Read the model definition and answer for the solid it produces. Units are mm, in the model's axes. A direction names the side the tool comes from. Round coordinates to 2 decimals unless told otherwise and drop trailing zeros. Write each loop counter-clockwise with the first axis right and the second up, starting at its lowest first coordinate (ties: lowest second). Pieces come first, ordered by that corner, then holes. Notation, with made-up numbers: (69, -27) -> (97, -27) arc R24 ccw to (97, -16) -> close; hole circle Ø9 at (0.5, 40). An arc over 180 degrees is marked (long way). Return JSON: item names as keys, results as strings.
from build123d import *

# Parameters (mm, degrees)
EXTRUDE_1_DEPTH              = 17.5
HOLE_WIZARD_M4_1_D           = 3.3
HOLE_WIZARD_M4_1_DEPTH       = 9.5
HOLE_WIZARD_M4_1_TIP         = 0.991420021
HOLE_WIZARD_M6_1_D           = 5
HOLE_WIZARD_M6_1_DEPTH       = 12
HOLE_WIZARD_M6_1_CSINK_D     = 6.05
HOLE_WIZARD_M6_1_CSINK_ANGLE = 90
HOLE_WIZARD_M6_1_TIP         = 1.502151548


with BuildPart() as part:
    # 草图1 → 凸台-拉伸1 (new, symmetric)
    with BuildSketch(Plane.XY):
        with BuildLine():
            Line((-27.5, 30), (27.5, 30))
            Line((27.5, 30), (27.5, -17))
            Line((27.5, -17), (9, -17))
            Line((9, -17), (9, -13.228756555))
            ThreePointArc((9, -13.228756555), (0, 16), (-9, -13.228756555))
            Line((-9, -13.228756555), (-9, -17))
            Line((-9, -17), (-27.5, -17))
            Line((-27.5, -17), (-27.5, 30))
        make_face()
    extrude(amount=EXTRUDE_1_DEPTH, both=True)

    # M4 螺纹孔1
    with Locations(Plane.XY.offset(17.5)):
        with Locations((18.186533479, 10.5), (18.186533479, -10.5), (-18.186533479, -10.5), (-18.186533479, 10.5)):
            Hole(HOLE_WIZARD_M4_1_D / 2, depth=HOLE_WIZARD_M4_1_DEPTH)
            with Locations((0, 0, -(HOLE_WIZARD_M4_1_DEPTH + HOLE_WIZARD_M4_1_TIP / 2))):  # 118° drill point
                Cone(0, HOLE_WIZARD_M4_1_D / 2, HOLE_WIZARD_M4_1_TIP, mode=Mode.SUBTRACT)

    # M6 螺纹孔1
    with Locations(Plane(origin=(-20.5, 30, 10.5), x_dir=(0, 0, 1), z_dir=(0, 1, 0))):
        with Locations((0, 0), (-21, 0), (-21, 41), (0, 41)):
            CounterSinkHole(HOLE_WIZARD_M6_1_D / 2, HOLE_WIZARD_M6_1_CSINK_D / 2, depth=HOLE_WIZARD_M6_1_DEPTH, counter_sink_angle=HOLE_WIZARD_M6_1_CSINK_ANGLE)
            with Locations((0, 0, -(HOLE_WIZARD_M6_1_DEPTH + HOLE_WIZARD_M6_1_TIP / 2))):  # 118° drill point
                Cone(0, HOLE_WIZARD_M6_1_D / 2, HOLE_WIZARD_M6_1_TIP, mode=Mode.SUBTRACT)


solid = part.part
Item 1: For a pull along X with two mould halves and no side action, classify faces 1 (the flat face through (0, 30, 0)), 2 (the cylindrical face through (-18.02, 23.66, 10.83)), 3 (the flat face through (-27.5, 6, 0)) as released by +X, released by -X, zero draft, split by the parting line, or undercut.
Worked answers:
{"face 1": "zero draft", "face 2": "undercut", "face 3": "released by -X"}
Item 2: Section A-A (y = 0) is taken. Give the vertices of the cut face in (x, z).
Worked answers:
{"outline": "(-27.5, -17.5) -> (-16, -17.5) -> (-16, 17.5) -> (-27.5, 17.5) -> close; (16, -17.5) -> (27.5, -17.5) -> (27.5, 17.5) -> (16, 17.5) -> close"}
Item 3: Section D-D (z = -14.5) is taken. Give the vertices of the cut face in (x, y), then the cut area to 3 significant figures.
Worked answers:
{"outline": "(-27.5, -17) -> (-9, -17) -> (-9, -13.23) arc R16 cw (long way) to (9, -13.23) -> (9, -17) -> (27.5, -17) -> (27.5, 30) -> (-27.5, 30) -> close", "area": "1,750 mm2"}
Item 4: Section B-B (y = 21) is taken. Give the vertices of the cut face in (x, z).
Worked answers:
{"outline": "(-27.5, -17.5) -> (27.5, -17.5) -> (27.5, 17.5) -> (-27.5, 17.5) -> close; hole circle Ø5 at (-20.5, -10.5); hole circle Ø5 at (-20.5, 10.5); hole circle Ø5 at (20.5, -10.5); hole circle Ø5 at (20.5, 10.5)"}
Item 5: Straight lines are drawn through the part: L1, parallel to Z at x = -20.5, y = 25.25; L2, parallel to X at y = 20.5, z = 10.5; L3, parallel to X at y = -11.5, z = 15.5. For each, find the intervals that lie inside material, in ascending order. Write a range as [from, to].
Worked answers:
{"L1": "z = [-17.5, -13], [-8, 8], [13, 17.5]", "L2": "x = [-27.5, -23], [-18, 18], [23, 27.5]", "L3": "x = [-27.5, -19.5], [-16.87, -11.12], [11.12, 16.87], [19.5, 27.5]"}
Item 6: A tool of negligible diameter and unlimited length cuts with its end or side. For faces 4 (the flat face through (9, -15, 0)), 5 (the cylindrical face through (22.98, 23.66, 10.83)), 6 (the flat face through (0, 17, 17.5)), 7 (the cylindrical face through (-19.71, 9.87, 12.68)), from which of +Z, -Z, +X, -X, +Y, -Y can it reach the whole face along a straight path? Write none if from no direction.
Worked answers:
{"face 4": "+Z, -Z, -Y", "face 5": "+Y", "face 6": "+Z, +X, -X, +Y, -Y", "face 7": "+Z"}
Item 7: Section C-C (x = 12.5) is taken. Give the vertices of the cut face in (y, z), then the cut area to 3 significant figures.
Worked answers:
{"outline": "(-17, -17.5) -> (-9.99, -17.5) -> (-9.99, 17.5) -> (-17, 17.5) -> close; (9.99, -17.5) -> (30, -17.5) -> (30, 17.5) -> (9.99, 17.5) -> close", "area": "946 mm2"}
Item 8: Flat-ended cylindrical pins translate along their axes: pin 1 (2 mm diameter, centred on x = 3, z = 1, fed in from -Y); pin 2 (4.5 mm diameter, centred on x = 18.19, y = -10.5, fed in from +Z). Find the tip coordinate at first contact, or state that the pin passes through.
Worked answers:
{"pin 1": "stops at y = 15.49", "pin 2": "stops at z = 17.5"}
